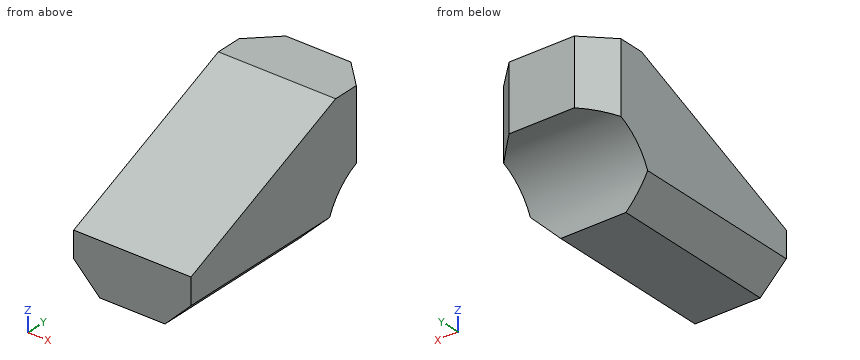
from build123d import *

# Parameters (mm, degrees)
BOSS_EXTRUDE1_DEPTH = 22.5
CHAMFER1_SIZE       = 10


with BuildPart() as part:
    # Sketch1 → Boss-Extrude1 (new, symmetric)
    with BuildSketch(Plane(origin=(0, 0, 0), x_dir=(0, 0, -1), z_dir=(1, 0, 0))):
        with BuildLine():
            Line((0, 0), (0, 65))
            ThreePointArc((0, 65), (-17.67766953, 72.32233047), (-25, 90))
            Line((-25, 90), (-50, 90))
            Line((-50, 90), (-50, 70))
            Line((-50, 70), (-20, 0))
            Line((-20, 0), (0, 0))
        make_face()
    extrude(amount=BOSS_EXTRUDE1_DEPTH, both=True)

    # Chamfer1
    chamfer1_edges = [part.edges().sort_by_distance(p)[0] for p in [
        (22.5, 90, 37.5),
        (-22.5, 90, 37.5),
        (22.5, 32.5, 0),
        (-22.5, 32.5, 0),
    ]]
    chamfer(chamfer1_edges, length=CHAMFER1_SIZE)


solid = part.part
Can you work these out from the model? Positions are in its coordinate system, mm. Give positions to 0.01 mm unless a question says otherwise; leave off trailing zeros. Order: outer loops, then holes, each group sorted by start corner. A loop starts at its lowest first (then second) coordinate and runs counter-clockwise, first axis right, second up. Notation, with made-up numbers: M -4,82.25 L 5,82.25 A16 cw 5,112.25 Z; hole C 74,48.5 d6. An arc over 180 degrees is marked long. Use one line per item in the form item = value. Start each with the question number.
Item 1: If we section it at C-C (y = 78): Write out the boundary of the cut face in (x, z), then the cut area to 3 significant figures.
Item 2: If I drill on line 1 along Z through (x, y) = (5, 39); line 2 along Z through (x, y) = (-1.5, 12); line 3 along Y through (x, z) = (-1.5, 48), over which ranges is the centre line in solid material (lowest first)?
Item 3: If we section it at B-B (y = 42): Write out the boundary of the cut face in (x, z).
Item 4: Will these pins go through, and if not, where does the flat tip stop? pin 1 Ø1 at (x, y) = (-9.5, 18.5) entering from +Z; pin 2 Ø2 at (y, z) = (27.5, 33.5) entering from -X; pin 3 Ø1 at (x, z) = (7.5, 14) entering from +Y.
Item 5: If we section it at A-A (z = 42.5): Write out the boundary of the cut face in (x, y), then the cut area to 3 significant figures.
Outcome:
q1.outline = M -22.5,21.93 L 22.5,21.93 L 22.5,50 L -22.5,50 Z
q1.area = 1,260 mm2
q2.line_1 = 0 to 36.71
q2.line_2 = 0 to 25.14
q2.line_3 = 65.33 to 90
q3.outline = M -22.5,10 L -12.5,0 L 12.5,0 L 22.5,10 L 22.5,38 L -22.5,38 Z
q4.pin_1 = 28.14
q4.pin_2 = through
q4.pin_3 = 69.63
q5.outline = M -22.5,52.5 L 22.5,52.5 L 22.5,80 L 12.5,90 L -12.5,90 L -22.5,80 Z
q5.area = 1,590 mm2
